Design review of the part built by this model. Coordinates are the model's own, in mm. A direction names the side the tool comes from. Give positions to 0.01 mm unless a question says otherwise; leave off trailing zeros. Loops run counter-clockwise (first coordinate to the right, second up) from the corner with the lowest first, then second, coordinate; pieces in that order, holes last. Notation, with made-up numbers: (17, -26) - (51, -26) arc R30 cw to (51, -1) - close; hole circle Ø1 at (60, 54). An arc over 180 degrees is marked (long way). Write each question's results on one line, items separated by ' | '.
from build123d import *

# Parameters (mm, degrees)
EXTRUDE_THIN1_DEPTH  = 276
EXTRUDE_THIN2_DEPTH  = 2
EXTRUDE_THIN3_DEPTH  = 2
CUT_EXTRUDE1_DEPTH   = 2
LPATTERN1_COUNT      = 2
LPATTERN1_PITCH      = 400
LPATTERN1_COUNT_DIR2 = 2
LPATTERN1_PITCH_DIR2 = 70
CUT_EXTRUDE2_DEPTH   = 2
LPATTERN2_COUNT      = 2
LPATTERN2_PITCH      = 70
SKETCH7_W            = 2
SKETCH7_H            = 276
BOSS_EXTRUDE1_DEPTH  = 10


with BuildPart() as part:
    # Sketch1 → Extrude-Thin1 (new body)
    with BuildSketch(Plane.XY):
        Polygon((-856.990015303, 38.44340597), (-712, 0), (0, 0), (0, 120), (-2, 120), (-2, 2), (-711.739357917, 2), (-856.477436556, 40.376606174), align=None)
    extrude(amount=EXTRUDE_THIN1_DEPTH)

    # Sketch2 → Extrude-Thin2 (add)
    with BuildSketch(Plane.XY.offset(276)):
        Polygon((0, 0), (-712, 0), (-856.990015303, 38.44340597), (-853.914542825, 50.042607194), (-710.436147504, 12), (0, 12), align=None)
    extrude(amount=EXTRUDE_THIN2_DEPTH)

    # Sketch4 → Extrude-Thin3 (add)
    with BuildSketch(Plane(origin=(0, 0, 0), x_dir=(-1, 0, 0), z_dir=(0, 0, -1))):
        Polygon((0, 0), (712, 0), (856.990015303, 38.44340597), (853.914542825, 50.042607194), (710.436147504, 12), (0, 12), align=None)
    extrude(amount=EXTRUDE_THIN3_DEPTH)

    # Sketch5 → Cut-Extrude1 (cut)
    with BuildSketch(Plane.XZ):
        with BuildLine():
            Line((-122.5, 254), (-107.5, 254))
            ThreePointArc((-107.5, 254), (-101.5, 248), (-107.5, 242))
            Line((-107.5, 242), (-122.5, 242))
            ThreePointArc((-122.5, 242), (-128.5, 248), (-122.5, 254))
        make_face()
    cut_extrude1 = extrude(amount=-CUT_EXTRUDE1_DEPTH, mode=Mode.SUBTRACT)

    # LPattern1: Cut-Extrude1 2 × 2
    with Locations(*[(-i * LPATTERN1_PITCH, 0, -j * LPATTERN1_PITCH_DIR2) for i in range(LPATTERN1_COUNT) for j in range(LPATTERN1_COUNT_DIR2) if (i, j) != (0, 0)]):
        add(cut_extrude1, mode=Mode.SUBTRACT)

    # Sketch6 → Cut-Extrude2 (cut)
    with BuildSketch(Plane(origin=(-46.76718086, -176.383285962, 0), x_dir=(0.9666001020169073, -0.2562893731329973, 0), z_dir=(-0.2562893731329973, -0.9666001020169073, 0))):
        with BuildLine():
            Line((-809.719272636, 254), (-794.719272636, 254))
            ThreePointArc((-794.719272636, 254), (-788.719272636, 248), (-794.719272636, 242))
            Line((-794.719272636, 242), (-809.719272636, 242))
            ThreePointArc((-809.719272636, 242), (-815.719272636, 248), (-809.719272636, 254))
        make_face()
    cut_extrude2 = extrude(amount=-CUT_EXTRUDE2_DEPTH, mode=Mode.SUBTRACT)

    # LPattern2: Cut-Extrude2 ×2
    with Locations(*[(0, 0, -i * LPATTERN2_PITCH) for i in range(1, LPATTERN2_COUNT)]):
        add(cut_extrude2, mode=Mode.SUBTRACT)

    # Sketch7 → Boss-Extrude1 (add)
    with BuildSketch(Plane(origin=(-46.254602114, -174.450085758, 0), x_dir=(0.9666001020169073, -0.25628937313299727, 0), z_dir=(0.25628937313299727, 0.9666001020169073, 0))):
        with Locations((-837.219272636, -138)):
            Rectangle(SKETCH7_W, SKETCH7_H)
    extrude(amount=BOSS_EXTRUDE1_DEPTH)


solid = part.part
(1) Tool access review of faces 4 (the flat face through (-426, 8, 278)), 5 (the flat face through (-426, 10, 276)): name each direction out of +Z, -Z, +X, -X, +Y, -Y from which nothing blocks a thin tool from reaching the whole face with its end or side.
Answers below:
face 4: +Z, +X, -X, +Y, -Y | face 5: +Y
(2) Take a section at C-C on y = 77. Give the boundary of the cut face in (x, z), plus the area to 3 significant figures.
Answers below:
outline: (-2, 0) - (0, 0) - (0, 276) - (-2, 276) - close | area: 552 mm2
(3) Take a section at B-B on z = 84. Give the boundary of the cut face in (x, y), plus the area to 3 significant figures.
Answers below:
outline: (-856.99, 38.44) - (-712, 0) - (0, 0) - (0, 120) - (-2, 120) - (-2, 2) - (-711.74, 2) - (-854.54, 39.86) - (-851.98, 49.53) - (-853.91, 50.04) - close | area: 1,980 mm2
(4) Draft analysis for pull direction X (two halves, no side actions). For faces 1 (the flat face through (-783.48, 18.953, 139.96)), 2 (the flat face through (-426, 8, -2)), 3 (the flat face through (-426, 10, 0)), state which applies: pulls with the +X half, pulls with the -X half, needs draft (parallel to the pull), parting line crosses it, or undercut.
Answers below:
face 1: pulls with the -X half | face 2: needs draft | face 3: undercut
(5) Wall thickness on line 1 along Y through (x, z) = (-151, 223.5); line 2 along X through (y, z) = (83, 158); line 3 along Z through (x, y) = (-186, 6): over which ranges is each line inside the solid? List them lowest first. Write a range as from..to.
Answers below:
line 1: 0..2 | line 2: -2..0 | line 3: -2..0, 276..278
(6) Take a section at A-A on x = -261.5. Give the boundary of the cut face in (y, z), plus the area to 3 significant figures.
Answers below:
outline: (0, -2) - (12, -2) - (12, 0) - (2, 0) - (2, 276) - (12, 276) - (12, 278) - (0, 278) - close | area: 600 mm2
(7) Insertion check: P1, Ø1.6, axis at x = -1.5, y = 77.5, coming from the -Z side; P2, Ø24, axis at x = -228.5, y = 31, coming from the -Z side; P3, Ø4, axis at y = 21, z = 132, coming from the +X side; P4, Ø4, axis at x = -126, z = 61.5, coming from the +Y side. Each pin has a flat end and moves straight along its axis. Give the tip position at first contact, or say it passes through.
Answers below:
P1: z = 0 | P2: through | P3: x = 0 | P4: y = 2
